Check sheet for the modelled part. Datum: model origin and axes. Units: mm. A direction names the side the tool comes from. Coordinates: 2 decimals unless noted, no trailing zeros. Loops run counter-clockwise (first coordinate to the right, second up) from the corner with the lowest first, then second, coordinate; pieces in that order, holes last. Notation, with made-up numbers: M -34.5,85.25 L -20.5,85.25 A32 cw -20.5,114.25 Z; hole C 53.5,84 d7. An arc over 180 degrees is marked long. Answer in a Markdown table with one row per item. Add a question column.
```python
from build123d import *

# Parameters (mm, degrees)
SKETCH1_R                                           = 38
BOSS_EXTRUDE1_DEPTH                                 = 10
SKETCH2_R                                           = 27.5
BOSS_EXTRUDE2_DEPTH                                 = 8
SKETCH3_R                                           = 23.5
CUT_EXTRUDE1_DEPTH                                  = 7
CUT_EXTRUDE2_START                                  = -7
SKETCH4_R                                           = 23.5
CUT_EXTRUDE2_DEPTH                                  = 7
SKETCH6_R                                           = 20
CUT_EXTRUDE3_DEPTH                                  = 57.674509261
CBORE_FOR_M5_HEX_SOCKET_HEAD_CAP_SCREW1_D           = 5.5
CBORE_FOR_M5_HEX_SOCKET_HEAD_CAP_SCREW1_CBORE_D     = 10
CBORE_FOR_M5_HEX_SOCKET_HEAD_CAP_SCREW1_CBORE_DEPTH = 5.4


with BuildPart() as part:
    # Sketch1 → Boss-Extrude1 (new body)
    with BuildSketch(Plane.XY):
        Circle(SKETCH1_R)
    extrude(amount=BOSS_EXTRUDE1_DEPTH)

    # Sketch2 → Boss-Extrude2 (add)
    with BuildSketch(Plane.XY.offset(10)):
        Circle(SKETCH2_R)
    extrude(amount=BOSS_EXTRUDE2_DEPTH)

    # Sketch3 → Cut-Extrude1 (cut)
    with BuildSketch(Plane.XY.offset(18)):
        Circle(SKETCH3_R)
    extrude(amount=-CUT_EXTRUDE1_DEPTH, mode=Mode.SUBTRACT)

    # Sketch4 → Cut-Extrude2 (cut)
    with BuildSketch(Plane(origin=(0, 0, 0), x_dir=(-1, 0, 0), z_dir=(0, 0, -1)).offset(CUT_EXTRUDE2_START)):
        with Locations(Location((0, 0, 0), (0, 0, 180))):
            Circle(SKETCH4_R)
    extrude(amount=CUT_EXTRUDE2_DEPTH, mode=Mode.SUBTRACT)

    # Sketch6 → Cut-Extrude3 (cut, through all)
    with BuildSketch(Plane.XY.offset(18)):
        Circle(SKETCH6_R)
    extrude(amount=-CUT_EXTRUDE3_DEPTH, mode=Mode.SUBTRACT)

    # CBORE for M5 Hex Socket Head Cap Screw1 (through all)
    with Locations(Plane(origin=(0, 0, 0), x_dir=(-1, 0, 0), z_dir=(0, 0, -1))):
        with Locations((0, 32.5), (-32.5, 0), (0, -32.5), (32.5, 0)):
            CounterBoreHole(CBORE_FOR_M5_HEX_SOCKET_HEAD_CAP_SCREW1_D / 2, CBORE_FOR_M5_HEX_SOCKET_HEAD_CAP_SCREW1_CBORE_D / 2, CBORE_FOR_M5_HEX_SOCKET_HEAD_CAP_SCREW1_CBORE_DEPTH)


solid = part.part
```
Q1. Cross-section at C-C (z = 9). Record the cut outline in (x, y), plus the area to 3 significant figures.
Q2. Thickness scan on L1, parallel to Y at x = 0, z = 2.35; L2, parallel to Y at x = 0, z = 6.75; L3, parallel to X at y = 0.5, z = 7.75. Record the ranges inside material, lowest first.
Q3. Cross-section at A-A (x = -32.5). Record the cut outline in (y, z), plus the area to 3 significant figures.
Q4. Access from +Z, -Z, +X, -X, +Y, -Y to the whole of each face (thin tool, end or side, straight path). Record for faces 1 (the face through (-5.961, -26.846, 13.944)), 2 (the face through (-17.4, -16.4, 0)), 3 (the face through (-35, -2, 5.4)).
Q5. Cross-section at B-B (y = 17). Record the cut outline in (x, z).
Q6. Cross-section at D-D (z = 15.75). Record the cut outline in (x, y), plus the area to 3 significant figures.
Q7. Go/stop test with flat-tipped pins: pin 1 (2 mm diameter, centred on y = 22, z = 6, fed in from -X); pin 2 (7 mm diameter, centred on x = 0, y = -32.5, fed in from -Z); pin 3 (6 mm diameter, centred on y = -12.5, z = 7.5, fed in from -X); pin 4 (3.5 mm diameter, centred on x = 32.5, y = 0, fed in from +Z). Record where each tip stops, or that it passes through.
Answer key:
| question | item | result |
|---|---|---|
| 1 | outline | C 0,0 d76; hole C -32.5,0 d5.5; hole C 0,0 d40; hole C 0,-32.5 d5.5; hole C 0,32.5 d5.5; hole C 32.5,0 d5.5 |
| 1 | area | 3,180 mm^2 |
| 2 | L1 | -38 to -37.5, -27.5 to -23.5, 23.5 to 27.5, 37.5 to 38 |
| 2 | L2 | -38 to -35.25, -29.75 to -23.5, 23.5 to 29.75, 35.25 to 38 |
| 2 | L3 | -38 to -35.2, -29.8 to -19.99, 19.99 to 29.8, 35.2 to 38 |
| 3 | outline | M -19.69,0 L -5,0 L -5,5.4 L -2.75,5.4 L -2.75,10 L -19.69,10 Z; M 2.75,5.4 L 5,5.4 L 5,0 L 19.69,0 L 19.69,10 L 2.75,10 Z |
| 3 | area | 315 mm^2 |
| 4 | face 1 | +Z |
| 4 | face 2 | -Z, +X, -X, +Y, -Y |
| 4 | face 3 | -Z |
| 5 | outline | M -33.99,0 L -16.22,0 L -16.22,7 L -10.54,7 L -10.54,11 L -16.22,11 L -16.22,18 L -21.62,18 L -21.62,10 L -33.99,10 Z; M 10.54,7 L 16.22,7 L 16.22,0 L 33.99,0 L 33.99,10 L 21.62,10 L 21.62,18 L 16.22,18 L 16.22,11 L 10.54,11 Z |
| 6 | outline | C 0,0 d55; hole C 0,0 d47 |
| 6 | area | 641 mm^2 |
| 7 | pin 1 | x = -31.67 |
| 7 | pin 2 | z = 5.4 |
| 7 | pin 3 | x = -36.79 |
| 7 | pin 4 | through |
